Here's the drawing with two shaded views (mm, measured from the low corner). I have some questions. A direction names the side the tool comes from. Give positions to 0.01 mm unless a question says otherwise; leave off trailing zeros. Order: outer loops, then holes, each group sorted by start corner. A loop starts at its lowest first (then second) coordinate and runs counter-clockwise, first axis right, second up. Notation, with made-up numbers: M 83,-8.5 L 129,-8.5 A29 cw 129,17.5 Z; hole C -17,84 d7. An arc over 180 degrees is marked long. Use a Markdown table: item, result. Add a question column.
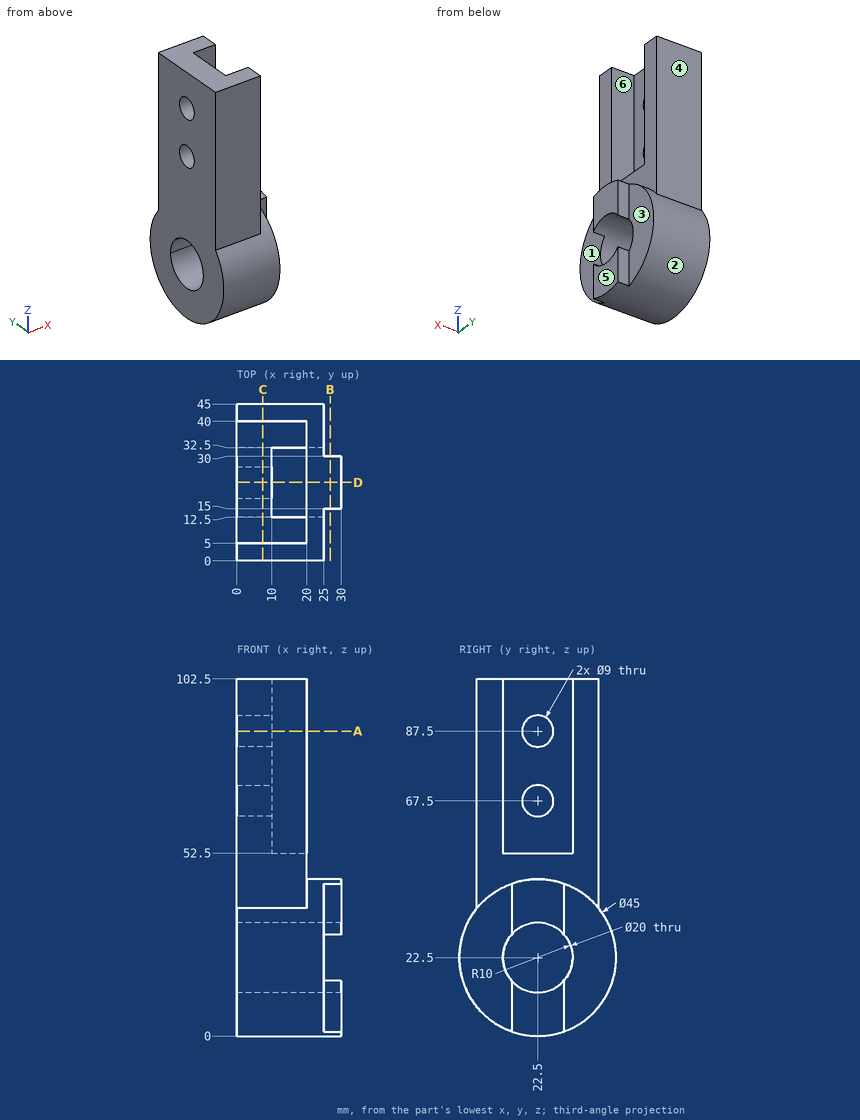
1. On a 3-axis mill with a long thin cutter (end or side, diameter ignored), from which of +Z, -Z, +X, -X, +Y, -Y can I reach the whole of each face in a straight line? I mean the marked faces 1, 2 and 3. Say none if no direction works.
2. If we section it at C-C, the plane x = 7.5: List the corners of the cut face in (y, z) for me, then the cut area to 3 significant figures.
3. We'd pull the mould along Y, two halves only. Please class the marked faces 4, 5 and 6: +Y half, -Y half, draft (parallel to the pull), parting line (faces both ways), or undercut.
4. Will these pins go through, and if not, where does the flat tip stop? pin 1 (12 mm diameter, centred on y = 40, z = 22, fed in from +X); pin 2 (10.5 mm diameter, centred on y = 21, z = 78.5, fed in from +X); pin 3 (1 mm diameter, centred on x = 4, z = 37.5, fed in from +Y); pin 4 (12 mm diameter, centred on y = 22.5, z = 22.5, fed in from -X).
5. If we section it at A-A, the plane z = 87.5: List the corners of the cut face in (x, y) for me, then the cut area to 3 significant figures.
6. I need wall thicknesses on L1, parallel to Y at x = 14, z = 62.5; L2, parallel to Y at x = 6, z = 87.5; L3, parallel to X at y = 32.5, z = 15. Which ranges of each line are inside material? Lowest first, please. Write a range as [from, to].
7. If we section it at D-D, the plane y = 22.5: List the corners of the cut face in (x, z) for me, then the cut area to 3 significant figures.
8. If we section it at B-B, the plane x = 26.75: List the corners of the cut face in (y, z) for me, then the cut area to 3 significant figures.
Geometry results:
| question | item | result |
|---|---|---|
| 1 | face 1 | +Z, -Z, +X, -Y |
| 1 | face 2 | +X |
| 1 | face 3 | +Z, -Z, +X, +Y |
| 2 | outline | M 5,36.64 A22.5 ccw long 40,36.64 L 40,102.5 L 5,102.5 Z; hole C 22.5,22.5 d20; hole C 22.5,67.5 d9; hole C 22.5,87.5 d9 |
| 2 | area | 3,250 mm^2 |
| 3 | face 4 | +Y half |
| 3 | face 5 | draft |
| 3 | face 6 | undercut |
| 4 | pin 1 | stops at x = 25 |
| 4 | pin 2 | stops at x = 10 |
| 4 | pin 3 | stops at y = 40 |
| 4 | pin 4 | passes through |
| 5 | outline | M 0,5 L 20,5 L 20,12.5 L 10,12.5 L 10,18 L 0,18 Z; M 0,27 L 10,27 L 10,32.5 L 20,32.5 L 20,40 L 0,40 Z |
| 5 | area | 410 mm^2 |
| 6 | L1 | y = [5, 12.5], [32.5, 40] |
| 6 | L2 | y = [5, 18], [27, 40] |
| 6 | L3 | x = [0, 25] |
| 7 | outline | M 0,0 L 30,0 L 30,12.5 L 0,12.5 Z; M 0,32.5 L 30,32.5 L 30,45 L 20,45 L 20,52.5 L 10,52.5 L 10,63 L 0,63 Z; M 0,72 L 10,72 L 10,83 L 0,83 Z; M 0,92 L 10,92 L 10,102.5 L 0,102.5 Z |
| 7 | area | 1,220 mm^2 |
| 8 | outline | M 15,1.29 A22.5 ccw 30,1.29 L 30,15.89 A10 cw 15,15.89 Z; M 15,29.11 A10 cw 30,29.11 L 30,43.71 A22.5 ccw 15,43.71 Z |
| 8 | area | 393 mm^2 |
